The figure shows three views and two pictorial views of one solid part (mm, origin at its lowest corner). Answer the questions. Coordinates: 2 decimals unless noted, no trailing zeros. Order: outer loops, then holes, each group sorted by start corner. A loop starts at its lowest first (then second) coordinate and runs counter-clockwise, first axis right, second up. Notation, with made-up numbers: (72, 72) -> (115, 72) arc R22 cw to (115, 82) -> close; hole circle Ø10 at (10.25, 39.25). An arc over 180 degrees is marked (long way). Return JSON: item names as keys, results as strings.
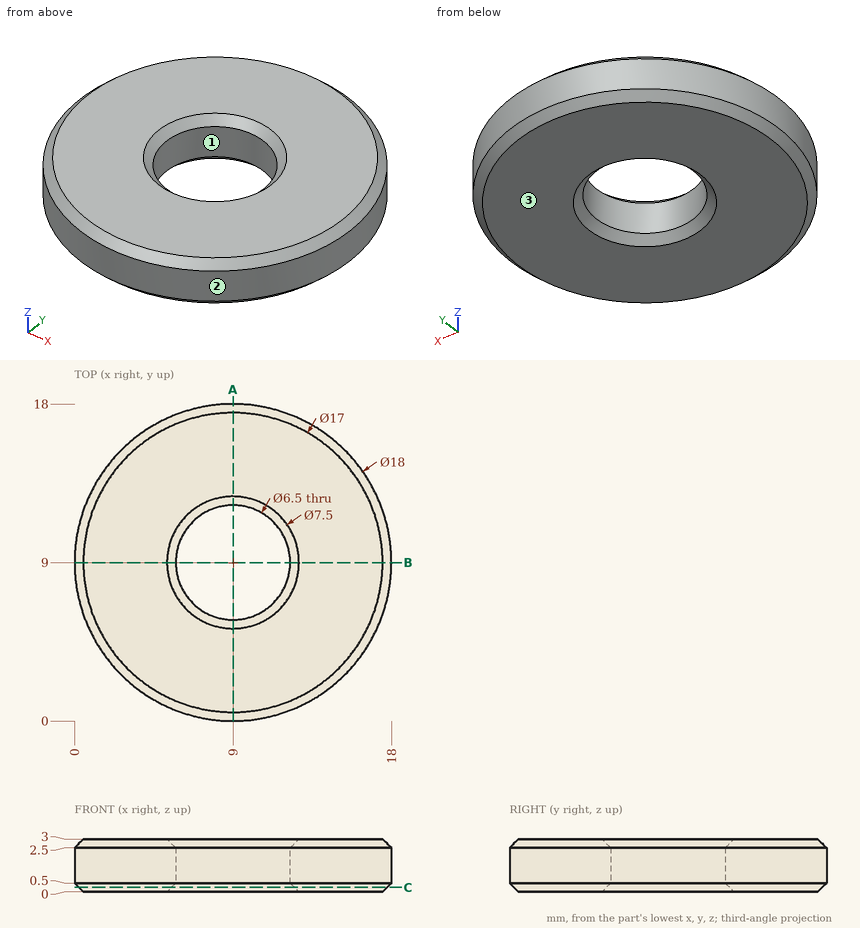
1. Consider line 1 (Y direction, x = 9, z = 1.1); line 2 (Y direction, x = 7.25, z = 0.85); line 3 (X direction, y = 11.5, z = 1.25). Determine where each line is inside the solid, lowest interval first. Write a range as from..to.
Answer block:
{"line 1": "y = 0..5.75, 12.25..18", "line 2": "y = 0.17..6.26, 11.74..17.83", "line 3": "x = 0.35..6.92, 11.08..17.65"}
2. Each of these flat-tipped pins is pushed along its axis until it touches: pin 1 Ø1 at (x, z) = (4.5, 2.5) entering from -Y; pin 2 Ø1.5 at (x, z) = (15, 1.5) entering from +Y. Where does it stop, or does it pass through?
Answer block:
{"pin 1": "stops at y = 0.94", "pin 2": "stops at y = 16.31"}
3. The part is cut by section C-C on z = 0.25. Give the vertices of the cut face in (x, y), and give its area (3 significant figures).
Answer block:
{"outline": "circle Ø17.5 at (9, 9); hole circle Ø7 at (9, 9)", "area": "202 mm2"}
4. The part is cut by section A-A on x = 9. Give the vertices of the cut face in (y, z), and give its area (3 significant figures).
Answer block:
{"outline": "(0, 0.5) -> (0.5, 0) -> (5.25, 0) -> (5.75, 0.5) -> (5.75, 2.5) -> (5.25, 3) -> (0.5, 3) -> (0, 2.5) -> close; (12.25, 0.5) -> (12.75, 0) -> (17.5, 0) -> (18, 0.5) -> (18, 2.5) -> (17.5, 3) -> (12.75, 3) -> (12.25, 2.5) -> close", "area": "33.5 mm2"}
5. Determine the mould class of the marked faces 1, 2 and 3 for opening direction X: pulls with the +X half, pulls with the -X half, needs draft (parallel to the pull), parting line crosses it, or undercut.
Answer block:
{"face 1": "undercut", "face 2": "parting line crosses it", "face 3": "needs draft"}
